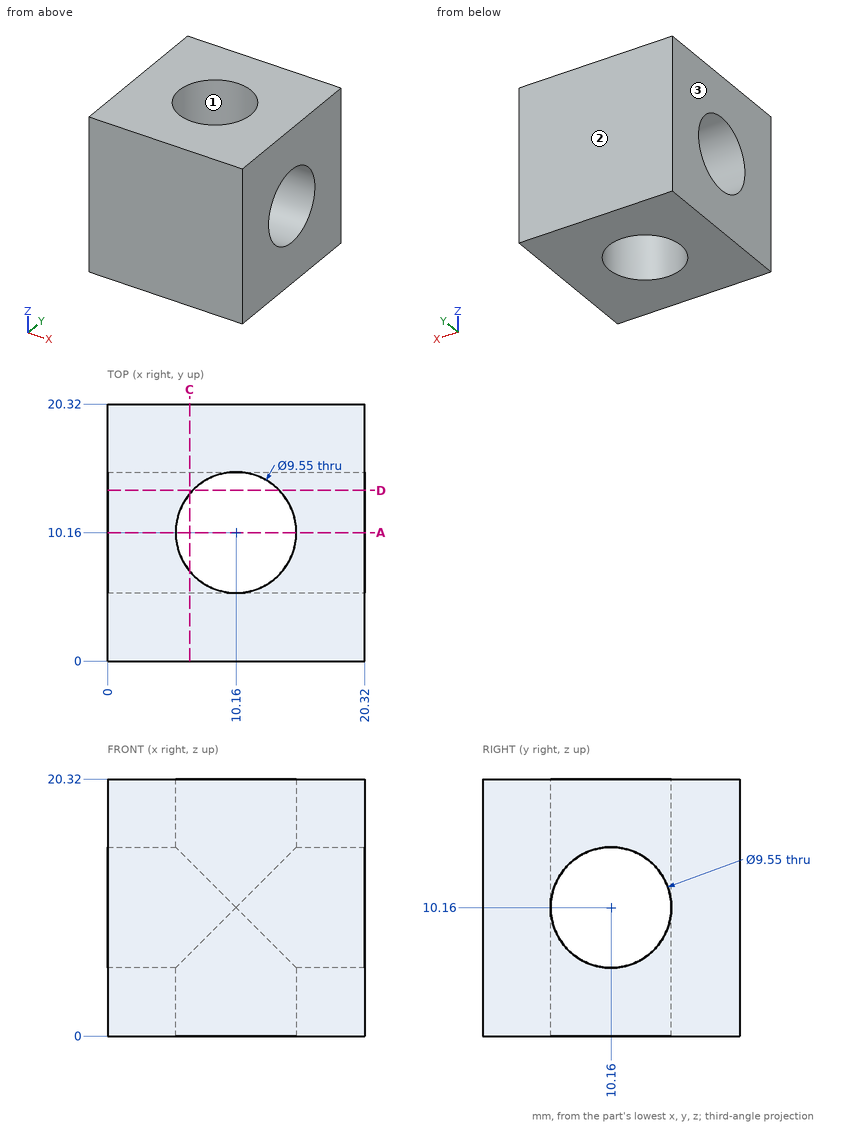
Here's the drawing with two shaded views (mm, measured from the low corner). I have some questions. Give positions to 0.01 mm unless a question says otherwise; leave off trailing zeros. Order: outer loops, then holes, each group sorted by start corner. A loop starts at its lowest first (then second) coordinate and runs counter-clockwise, first axis right, second up. Notation, with made-up numbers: M 29,79.5 L 61,79.5 A27 ccw 61,98.5 Z; hole C 72,53 d7. An arc over 180 degrees is marked long. One line per question, with ' | ' between items.
Item 1: Suppose I cut it at A-A, the plane y = 10.16. Write out the boundary of the cut face in (x, z) (3 decimals), then the cut area to 3 significant figures.
Answer block:
outline: M 0,0 L 5.385,0 L 5.385,5.385 L 0,5.385 Z; M 0,14.935 L 5.385,14.935 L 5.385,20.32 L 0,20.32 Z; M 14.935,0 L 20.32,0 L 20.32,5.385 L 14.935,5.385 Z; M 14.935,14.935 L 20.32,14.935 L 20.32,20.32 L 14.935,20.32 Z | area: 116 mm2
Item 2: Please list where these lines run through material, in increasing order: L1, parallel to Y at x = 10.16, z = 2.5 (3 decimals); L2, parallel to Y at x = 8, z = 16.25.
Answer block:
L1: y = 0 to 5.385, 14.935 to 20.32 | L2: y = 0 to 5.9, 14.42 to 20.32
Item 3: Suppose I cut it at C-C, the plane x = 6.5. Write out the boundary of the cut face in (y, z) (3 decimals), then the cut area to 3 significant figures.
Answer block:
outline: M 0,0 L 7.093,0 L 7.093,6.5 A4.775 cw 7.093,13.82 L 7.093,20.32 L 0,20.32 Z; M 13.227,0 L 20.32,0 L 20.32,20.32 L 13.227,20.32 L 13.227,13.82 A4.775 cw 13.227,6.5 Z | area: 271 mm2
Item 4: We'd pull the mould along X, two halves only. Please class the marked faces 1, 2 and 3: released by +X, released by -X, zero draft, split by the parting line, or undercut.
Answer block:
face 1: undercut | face 2: zero draft | face 3: released by -X
Item 5: Suppose I cut it at D-D, the plane y = 13.5. Write out the boundary of the cut face in (x, z).
Answer block:
outline: M 0,0 L 6.75,0 L 6.75,6.75 L 0,6.75 Z; M 0,13.57 L 6.75,13.57 L 6.75,20.32 L 0,20.32 Z; M 13.57,0 L 20.32,0 L 20.32,6.75 L 13.57,6.75 Z; M 13.57,13.57 L 20.32,13.57 L 20.32,20.32 L 13.57,20.32 Z
